For this review, use the dimensioned drawing (mm, ordinates from the lowest corner) and the shaded views. Coordinates: 2 decimals unless noted, no trailing zeros. Loops run counter-clockwise (first coordinate to the right, second up) from the corner with the lowest first, then second, coordinate; pieces in that order, holes last. Notation, with made-up numbers: (-29.75, 82.5) - (-20.75, 82.5) arc R25 cw to (-20.75, 96.5) - close; hole circle Ø3 at (-37, 78.25). An arc over 180 degrees is marked (long way). Return JSON: item names as keys, results as strings. Group by question number.
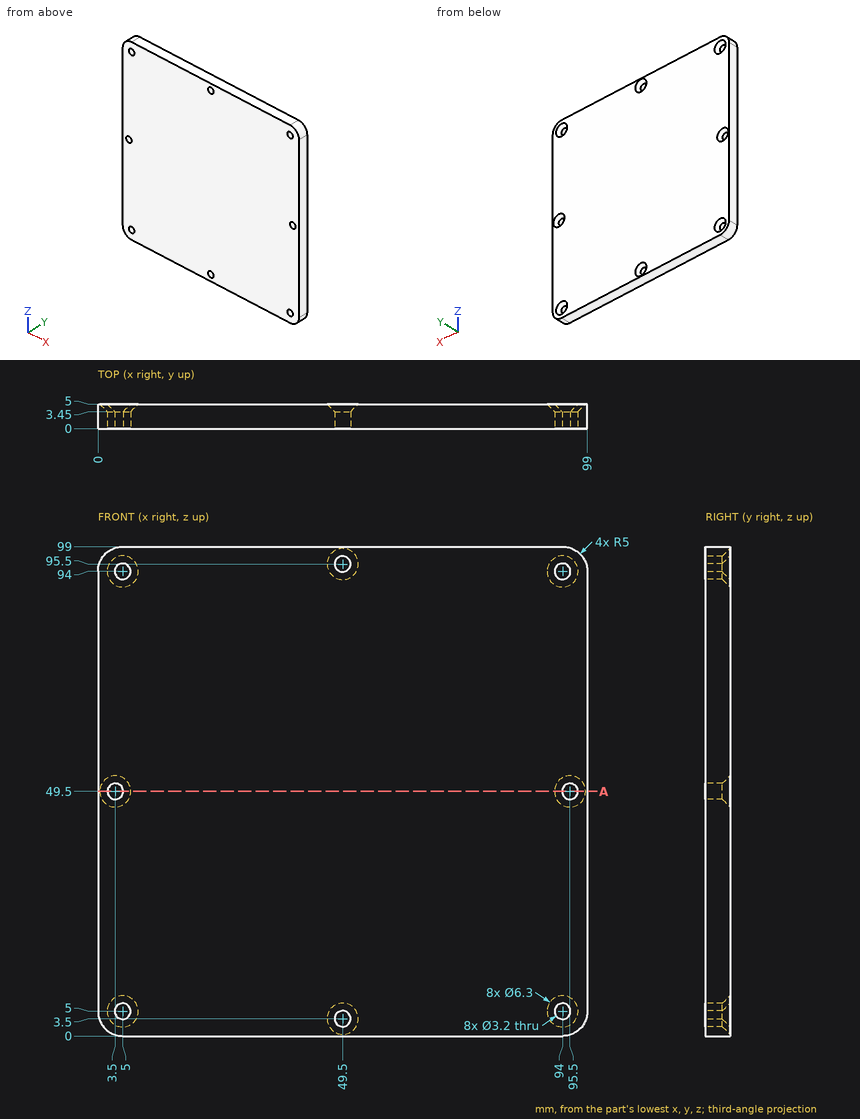
Item 1: Add section A-A (z = 49.5). State the section outline as (x, y) points, then the cut area to 3 significant figures.
Item 2: To check wall thickness, follow line 1 (X direction, y = 1.15, z = 49.5); line 2 (Z direction, x = 6, y = 1.5). State the ranges of each line that lie inside material, in increasing order. Write a range as from..to.
Item 3: For P1, Ø3.5, axis at x = 94, z = 5, coming from the +Y side; P2, Ø2.5, axis at x = 49.5, z = 95.5, coming from the -Y side, all flat-tipped, find the tip position at first contact; note any pin that passes through.
Answers below:
{
 "1": {"outline": "(0, 0) - (1.9, 0) - (1.9, 3.45) - (0.35, 5) - (0, 5) - close; (5.1, 0) - (93.9, 0) - (93.9, 3.45) - (92.35, 5) - (6.65, 5) - (5.1, 3.45) - close; (97.1, 0) - (99, 0) - (99, 5) - (98.65, 5) - (97.1, 3.45) - close", "area": "458 mm^2"},
 "2": {"line 1": "x = 0..1.9, 5.1..93.9, 97.1..99", "line 2": "z = 0..3.75, 6.25..92.75, 95.25..99"},
 "3": {"P1": "stops at y = 3.6", "P2": "passes through"}
}
